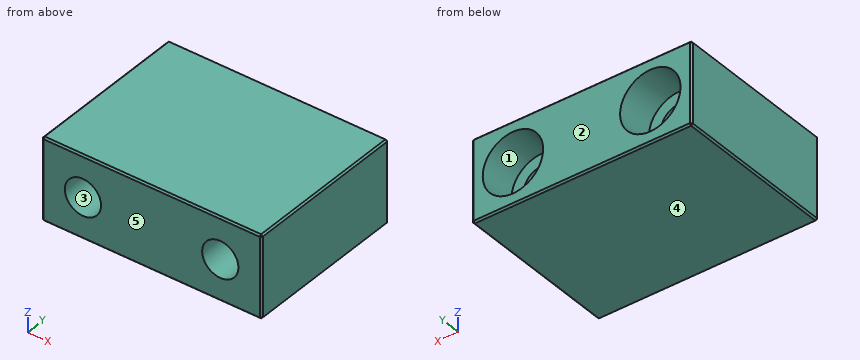
```python
from build123d import *

# Parameters (mm, degrees)
SKETCH_1_W                = 40
SKETCH_1_H                = 30
EXTRUDE_1_DEPTH           = 15
HOLE_WIZARD_1_D           = 6.6
HOLE_WIZARD_1_CBORE_D     = 11
HOLE_WIZARD_1_CBORE_DEPTH = 6.8
CHAMFER_1_SIZE            = 0.3


with BuildPart() as part:
    # 草图1 → 凸台-拉伸1 (new body)
    with BuildSketch(Plane.XY):
        Rectangle(SKETCH_1_W, SKETCH_1_H)
    extrude(amount=EXTRUDE_1_DEPTH)

    # 打孔尺寸根据内六角圆柱头螺钉的类型1 (through all)
    with Locations(Plane(origin=(0, 15, 0), x_dir=(1, 0, 0), z_dir=(0, 1, 0))):
        with Locations((-12.5, -7.5), (12.5, -7.5)):
            CounterBoreHole(HOLE_WIZARD_1_D / 2, HOLE_WIZARD_1_CBORE_D / 2, HOLE_WIZARD_1_CBORE_DEPTH)

    # 倒角1
    chamfer_1_edges = [part.edges().sort_by_distance(p)[0] for p in [
        (-20, 0, 15),
        (0, -15, 15),
        (20, 0, 15),
        (0, -15, 0),
        (-20, 0, 0),
        (0, 15, 0),
        (20, 0, 0),
        (0, 15, 15),
        (20, -15, 7.5),
        (-20, -15, 7.5),
        (-20, 15, 7.5),
        (20, 15, 7.5),
    ]]
    chamfer(chamfer_1_edges, length=CHAMFER_1_SIZE)


solid = part.part
```
Source: CAD feature listing. Evaluate the final solid. Frame: model axes, mm. Face numbers are marked on the shaded views. A direction names the side the tool comes from. Round coordinates to 2 decimals unless told otherwise and drop trailing zeros. Loops run counter-clockwise (first coordinate to the right, second up) from the corner with the lowest first, then second, coordinate; pieces in that order, holes last.
1. Section query C-C on y = 10.5. Output: boundary loops of the cut face in (x, z), and give its area (3 significant figures).
2. Section query B-B on z = 7.5. Output: boundary loops of the cut face in (x, y).
3. Ray query, L1, parallel to Z at x = 12.5, y = 12; L2, parallel to X at y = -13, z = 8; L3, parallel to X at y = 2, z = 9. Return the intervals inside material, ascending.
4. Contact query for flat-ended pins moving along their axis: pin 1 (4 mm diameter, centred on x = -12.5, z = 7.5, fed in from +Y); pin 2 (3.5 mm diameter, centred on x = 14.5, z = 5.5, fed in from +Y). Output: stop coordinate, or through.
5. Section query A-A on x = -12.5. Output: boundary loops of the cut face in (y, z), and give its area (3 significant figures).
6. Section query D-D on x = 13.5. Output: boundary loops of the cut face in (y, z).
7. Access query for the marked faces 1 and 2. Directions: +Z, -Z, +X, -X, +Y, -Y. A direction counts if a zero-diameter tool reaches every point of the face in a straight line with its end or side. Return the directions, or none.
8. Mould query, pull axis Z, two halves, no side actions, for the marked faces 3, 4 and 5. Classes: released by +Z, released by -Z, zero draft, split by the parting line, or undercut.
Answers below:
1. outline: (-20, 0.3) - (-19.7, 0) - (19.7, 0) - (20, 0.3) - (20, 14.7) - (19.7, 15) - (-19.7, 15) - (-20, 14.7) - close; hole circle Ø11 at (-12.5, 7.5); hole circle Ø11 at (12.5, 7.5)
1. area: 410 mm2
2. outline: (-20, -14.7) - (-19.7, -15) - (-15.8, -15) - (-15.8, 8.2) - (-18, 8.2) - (-18, 15) - (-19.7, 15) - (-20, 14.7) - close; (-9.2, -15) - (9.2, -15) - (9.2, 8.2) - (7, 8.2) - (7, 15) - (-7, 15) - (-7, 8.2) - (-9.2, 8.2) - close; (15.8, -15) - (19.7, -15) - (20, -14.7) - (20, 14.7) - (19.7, 15) - (18, 15) - (18, 8.2) - (15.8, 8.2) - close
3. L1: z = 0 to 2, 13 to 15
3. L2: x = -20 to -15.76, -9.24 to 9.24, 15.76 to 20
3. L3: x = -20 to -15.44, -9.56 to 9.56, 15.44 to 20
4. pin 1: passes through
4. pin 2: stops at y = 8.2
5. outline: (-15, 0.3) - (-14.7, 0) - (14.7, 0) - (15, 0.3) - (15, 2) - (8.2, 2) - (8.2, 4.2) - (-15, 4.2) - close; (-15, 10.8) - (8.2, 10.8) - (8.2, 13) - (15, 13) - (15, 14.7) - (14.7, 15) - (-14.7, 15) - (-15, 14.7) - close
5. area: 222 mm2
6. outline: (-15, 0.3) - (-14.7, 0) - (14.7, 0) - (15, 0.3) - (15, 2.09) - (8.2, 2.09) - (8.2, 4.36) - (-15, 4.36) - close; (-15, 10.64) - (8.2, 10.64) - (8.2, 12.91) - (15, 12.91) - (15, 14.7) - (14.7, 15) - (-14.7, 15) - (-15, 14.7) - close
7. face 1: +Y
7. face 2: +Z, -Z, +X, -X, +Y
8. face 3: undercut
8. face 4: released by -Z
8. face 5: zero draft
